from build123d import *

# Parameters (mm, degrees)
SKETCH1_W             = 70
SKETCH1_H             = 10
BOSS_EXTRUDE1_DEPTH   = 2
SKETCH2_W             = 20
SKETCH2_H             = 2
BOSS_EXTRUDE2_DEPTH   = 15
SKETCH3_W             = 20
SKETCH3_H             = 2
BOSS_EXTRUDE3_DEPTH   = 8
FILLET2_R             = 1
FILLET3_R             = 3
SKETCH4_R             = 2.25
CUT_EXTRUDE1_DEPTH    = 8
SKETCH6_W             = 7
SKETCH6_H             = 2
BOSS_EXTRUDE4_DEPTH   = 8
FILLET4_R             = 1
M3_TAPPED_HOLE1_D     = 2.5
M3_TAPPED_HOLE1_DEPTH = 7.5
M3_TAPPED_HOLE1_TIP   = 0.751075774
FILLET5_R             = 1


with BuildPart() as part:
    # Sketch1 → Boss-Extrude1 (new body)
    with BuildSketch(Plane.XY):
        Rectangle(SKETCH1_W, SKETCH1_H)
    extrude(amount=BOSS_EXTRUDE1_DEPTH)

    # Sketch2 → Boss-Extrude2 (add)
    with BuildSketch(Plane.XY.offset(2)):
        with Locations((0, 4)):
            Rectangle(SKETCH2_W, SKETCH2_H)
    extrude(amount=BOSS_EXTRUDE2_DEPTH)

    # Sketch3 → Boss-Extrude3 (add)
    with BuildSketch(Plane(origin=(0, 3, 0), x_dir=(-1, 0, 0), z_dir=(0, -1, 0))):
        with Locations((0, -16)):
            Rectangle(SKETCH3_W, SKETCH3_H)
    extrude(amount=BOSS_EXTRUDE3_DEPTH)

    # Fillet2
    fillet2_edges = [part.edges().sort_by_distance(p)[0] for p in [
        (0, 3, 2),
        (0, 3, 15),
    ]]
    fillet(fillet2_edges, radius=FILLET2_R)

    # Fillet3
    fillet3_edges = [part.edges().sort_by_distance(p)[0] for p in [
        (0, 5, 17),
    ]]
    fillet(fillet3_edges, radius=FILLET3_R)

    # Sketch4 → Cut-Extrude1 (cut)
    with BuildSketch(Plane.XY.offset(2)):
        with Locations((-30, 0)):
            Circle(SKETCH4_R)
        with Locations((30, 0)):
            Circle(SKETCH4_R)
    extrude(amount=-CUT_EXTRUDE1_DEPTH, mode=Mode.SUBTRACT)

    # Sketch6 → Boss-Extrude4 (add)
    with BuildSketch(Plane(origin=(0, -5, 0), x_dir=(-1, 0, 0), z_dir=(0, -1, 0))):
        with Locations((-17.5, -1)):
            Rectangle(SKETCH6_W, SKETCH6_H)
        with Locations((17.5, -1)):
            Rectangle(SKETCH6_W, SKETCH6_H)
    extrude(amount=BOSS_EXTRUDE4_DEPTH)

    # Fillet4
    fillet4_edges = [part.edges().sort_by_distance(p)[0] for p in [
        (35, -5, 1),
        (-35, -5, 1),
        (-35, 5, 1),
        (35, 5, 1),
    ]]
    fillet(fillet4_edges, radius=FILLET4_R)

    # M3 Tapped Hole1
    with Locations(Plane(origin=(-17.5, -9.5, 2), x_dir=(1, 0, 0), z_dir=(0, 0, 1))):
        with Locations((0, 0), (35, 0)):
            Hole(M3_TAPPED_HOLE1_D / 2, depth=M3_TAPPED_HOLE1_DEPTH)
            with Locations((0, 0, -(M3_TAPPED_HOLE1_DEPTH + M3_TAPPED_HOLE1_TIP / 2))):  # 118° drill point
                Cone(0, M3_TAPPED_HOLE1_D / 2, M3_TAPPED_HOLE1_TIP, mode=Mode.SUBTRACT)

    # Fillet5
    fillet5_edges = [part.edges().sort_by_distance(p)[0] for p in [
        (14, -5, 1),
        (21, -5, 1),
        (14, -13, 1),
        (21, -13, 1),
        (-21, -5, 1),
        (-14, -5, 1),
        (-21, -13, 1),
        (-14, -13, 1),
    ]]
    fillet(fillet5_edges, radius=FILLET5_R)


solid = part.part
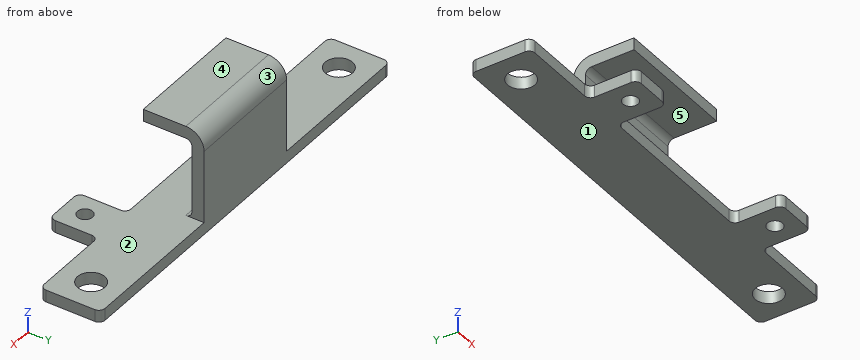
The listing builds one solid part. Answer for the finished solid, in the listing's coordinates (mm). Face numbers are marked on the shaded views. A direction names the side the tool comes from. Coordinates: 2 decimals unless noted, no trailing zeros. Order: outer loops, then holes, each group sorted by start corner. A loop starts at its lowest first (then second) coordinate and runs counter-clockwise, first axis right, second up. Notation, with made-up numbers: (11, 22) -> (41, 22) arc R16 cw to (41, 40) -> close; hole circle Ø10 at (60, 75). An arc over 180 degrees is marked (long way). Answer in a Markdown table with one row per item. Add a question column.
Item 1: Find section B-B (y = -9.5). Write down the section's boundary in (x, z).
Item 2: Find section C-C (x = 30). Write down the section's boundary in (y, z), then the cut area to 3 significant figures.
Item 3: Find the intervals of material crossed by L1, parallel to Y at x = 17.5, z = 1.2; L2, parallel to Y at x = -30, z = 1.5; L3, parallel to Z at x = 0.5, y = -4, in increasing order. Write a range as from..to.
Item 4: Find section A-A (x = 17.5). Write down the section's boundary in (y, z), then the cut area to 3 significant figures.
Item 5: Each of these flat-tipped pins is pushed along its axis until it touches: P1, Ø2, axis at y = -9, z = 0.5, coming from the -X side; P2, Ø5, axis at y = 1, z = 7.5, coming from the +X side; P3, Ø3, axis at x = 17.5, y = -9.5, coming from the -Z side; P4, Ø1, axis at y = -10, z = 1.5, coming from the +X side. Where does it stop, or does it pass through?
Item 6: Which of the six approach directions +Z, -Z, +X, -X, +Y, -Y give full straight-line access (tool end or side, diameter ignored) to the marked faces 4 and 5?
Item 7: Determine the mould class of the marked faces 1, 2 and 3 for opening direction Z: +Z half, -Z half, draft (parallel to the pull), parting line (faces both ways), or undercut.
Item 8: Find section D-D (y = 0). Write down the section's boundary in (x, z).
Result set:
| question | item | result |
|---|---|---|
| 1 | outline | (-21, 0) -> (-18.75, 0) -> (-18.75, 2) -> (-21, 2) -> close; (-16.25, 0) -> (-14, 0) -> (-14, 2) -> (-16.25, 2) -> close; (14, 0) -> (16.25, 0) -> (16.25, 2) -> (14, 2) -> close; (18.75, 0) -> (21, 0) -> (21, 2) -> (18.75, 2) -> close |
| 2 | outline | (-5, 0) -> (-2.25, 0) -> (-2.25, 2) -> (-5, 2) -> close; (2.25, 0) -> (5, 0) -> (5, 2) -> (2.25, 2) -> close |
| 2 | area | 11.0 mm² |
| 3 | L1 | y = -13..-10.75, -8.25..5 |
| 3 | L2 | y = -5..-2.25, 2.25..5 |
| 3 | L3 | z = 0..2, 15..17 |
| 4 | outline | (-13, 0) -> (-10.75, 0) -> (-10.75, 2) -> (-13, 2) -> close; (-8.25, 0) -> (5, 0) -> (5, 2) -> (-8.25, 2) -> close |
| 4 | area | 31.0 mm² |
| 5 | P1 | stops at x = -21 |
| 5 | P2 | stops at x = 10 |
| 5 | P3 | stops at z = 0 |
| 5 | P4 | stops at x = 21 |
| 6 | face 4 | +Z, +X, -X, +Y, -Y |
| 6 | face 5 | +X, -X, -Y |
| 7 | face 1 | -Z half |
| 7 | face 2 | undercut |
| 7 | face 3 | +Z half |
| 8 | outline | (-35, 0) -> (-32.25, 0) -> (-32.25, 2) -> (-35, 2) -> close; (-27.75, 0) -> (27.75, 0) -> (27.75, 2) -> (-27.75, 2) -> close; (-10, 15) -> (10, 15) -> (10, 17) -> (-10, 17) -> close; (32.25, 0) -> (35, 0) -> (35, 2) -> (32.25, 2) -> close |
